from build123d import *

# Parameters (mm, degrees)
BOSS_EXTRUDE1_DEPTH = 341
SKETCH2_R           = 10.5
CUT_EXTRUDE1_DEPTH  = 95


with BuildPart() as part:
    # Sketch1 → Boss-Extrude1 (new, symmetric)
    with BuildSketch(Plane(origin=(0, 0, 0), x_dir=(1, 0, 0), z_dir=(0, 1, 0))):
        Polygon((0, -37.5), (0, 37.5), (10, 42.881796684), (65, 60), (65, 45), (30, 35), (30, -35), (65, -45), (65, -60), (10, -42.881796684), align=None)
    extrude(amount=BOSS_EXTRUDE1_DEPTH, both=True)

    # Sketch2 → Cut-Extrude1 (cut)
    with BuildSketch(Plane.ZY):
        Circle(SKETCH2_R)
    extrude(amount=-CUT_EXTRUDE1_DEPTH, mode=Mode.SUBTRACT)


solid = part.part
CAD build for the part. Positions are in the model's coordinates, mm. A direction names the side the tool comes from. Coordinates: 2 decimals unless noted, no trailing zeros. Loops run counter-clockwise (first coordinate to the right, second up) from the corner with the lowest first, then second, coordinate; pieces in that order, holes last. Notation, with made-up numbers: (-29.5, 10.25) -> (9.5, 10.25) arc R23 cw to (9.5, 32.25) -> close; hole circle Ø10 at (24, 21.5). An arc over 180 degrees is marked (long way). One line per item, written item: value.
1. Slice it at D-D on y = -261. Write the cut outline in (x, z), and give its area (3 significant figures).
Answers:
outline: (0, -37.5) -> (10, -42.88) -> (65, -60) -> (65, -45) -> (30, -35) -> (30, 35) -> (65, 45) -> (65, 60) -> (10, 42.88) -> (0, 37.5) -> close
area: 3,660 mm^2
2. Slice it at B-B on y = 0. Write the cut outline in (x, z).
Answers:
outline: (0, -37.5) -> (10, -42.88) -> (65, -60) -> (65, -45) -> (30, -35) -> (30, -10.5) -> (0, -10.5) -> close; (0, 10.5) -> (30, 10.5) -> (30, 35) -> (65, 45) -> (65, 60) -> (10, 42.88) -> (0, 37.5) -> close
3. Flat gauge pins, fed straight in: P1, Ø2, axis at x = 54, z = 40, coming from the +Y side; P2, Ø3, axis at x = 27, y = 272, coming from the -Z side; P3, Ø3, axis at x = 17.5, y = -104, coming from the -Z side; P4, Ø1, axis at x = 55.5, y = -209.5, coming from the -Z side. Where does each tip first touch, or does it go through?
Answers:
P1: passes through
P2: stops at z = -48.64
P3: stops at z = -45.68
P4: stops at z = -57.2
4. Drill centre lines: line 1 (Y direction, x = 12, z = 0); line 2 (X direction, y = -112, z = 11); line 3 (Y direction, x = 18, z = 6). Where is each one in solid material? Low to high. Write a range as [from, to].
Answers:
line 1: y = [-341, -10.5], [10.5, 341]
line 2: x = [0, 30]
line 3: y = [-341, -8.62], [8.62, 341]
5. Slice it at A-A on z = 0. Write the cut outline in (x, y), and give its area (3 significant figures).
Answers:
outline: (0, -341) -> (30, -341) -> (30, -10.5) -> (0, -10.5) -> close; (0, 10.5) -> (30, 10.5) -> (30, 341) -> (0, 341) -> close
area: 19,800 mm^2
6. Slice it at C-C on x = 46. Write the cut outline in (y, z).
Answers:
outline: (-341, -54.09) -> (341, -54.09) -> (341, -39.57) -> (-341, -39.57) -> close; (-341, 39.57) -> (341, 39.57) -> (341, 54.09) -> (-341, 54.09) -> close
7. Which spindle directions (+Z, -Z, +X, -X, +Y, -Y) get a long thin tool onto all of the face, cutting with end or side? Do faces 5 (the face through (0, 5, -16)), 6 (the face through (47.26, 4.77, 39.93)). Say none if no direction does.
Answers:
face 5: +Z, -Z, -X, +Y, -Y
face 6: +X, +Y, -Y
8. Pull direction Z, two halves, no side cores. Call faces 1 (the face through (37.115, 4.774, -51.321)), 2 (the face through (47.74, 4.77, -40.07)), 3 (the face through (37.88, 4.77, 51.56)), 4 (the face through (30, 5, 15)): pulls with the +Z half, pulls with the -Z half, needs draft (parallel to the pull), parting line crosses it, or undercut.
Answers:
face 1: pulls with the -Z half
face 2: undercut
face 3: pulls with the +Z half
face 4: undercut
